Check sheet for the modelled part. Datum: model origin and axes. Units: mm. A direction names the side the tool comes from. Coordinates: 2 decimals unless noted, no trailing zeros. Loops run counter-clockwise (first coordinate to the right, second up) from the corner with the lowest first, then second, coordinate; pieces in that order, holes last. Notation, with made-up numbers: (2, 5.25) - (8, 5.25) arc R15 ccw to (8, 12.25) - close; hole circle Ø9 at (89.5, -34.5). An arc over 180 degrees is marked (long way). Write each question's results on one line, items separated by ' | '. Start each with the question number.
1. Gauge pin test, flat ends, axial feed: P1, Ø5, axis at y = -1.5, z = 24, coming from the +X side; P2, Ø2, axis at x = 0.5, z = -4.5, coming from the +Y side; P3, Ø3, axis at y = 4, z = 42.5, coming from the -X side; P4, Ø1.5, axis at y = 2.5, z = 8.5, coming from the -X side. Record the tip position at first contact, or that the pin passes through.
2. Tool access check on faces 1 (the face through (3, 0, 38)), 2 (the face through (2.175, -1.233, -4.768)), 3 (the face through (1.08, 4.88, -2.71)). Record the directions out of +Z, -Z, +X, -X, +Y, -Y that give a thin tool (end or side, any length) a straight path to the whole face; none if there is none.
3. Thickness scan on line 1 (Z direction, x = 1.75, y = -3.25); line 2 (Z direction, x = -1.75, y = 0.25); line 3 (X direction, y = -0.25, z = 3). Record the ranges inside material, lowest first. Write a range as [from, to].
4. Cross-section at B-B (z = 12.5). Record the cut outline in (x, y).
```python
from build123d import *

# Parameters (mm, degrees)
CUT_EXTRUDE1_DEPTH = 2.5


with BuildPart() as part:
    # Logo3_bib1 → Revolve1 (revolve)
    with BuildSketch(Plane(origin=(0, 0, 0), x_dir=(-1, 0, 0), z_dir=(0, -1, 0))):
        with BuildLine():
            Line((0, -50), (0, 6))
            Line((0, 6), (4.5, 6))
            ThreePointArc((4.5, 6), (4.853553391, 5.853553391), (5, 5.5))
            Line((5, 5.5), (5, 0))
            Line((5, 0), (3, 0))
            Line((3, 0), (3, -26.01))
            Line((3, -26.01), (2.613425636, -26.01))
            ThreePointArc((2.613425636, -26.01), (2.593729481, -26.026527036), (2.606585234, -26.048793852))
            Line((2.606585234, -26.048793852), (3, -26.191985117))
            Line((3, -26.191985117), (3, -49.5))
            Line((3, -49.5), (2.5, -50))
            Line((2.5, -50), (0, -50))
        make_face()
    revolve(axis=Axis((0, 0, -10.585154653), (0, 0, 1)))

    # Logo3_bib2 → Cut-Extrude1 (cut)
    with BuildSketch(Plane(origin=(0, 0, -6), x_dir=(1, 0, 0), z_dir=(0, 0, -1))):
        Polygon((2.886751346, 0), (1.443375673, 2.5), (-1.443375673, 2.5), (-2.886751346, 0), (-1.443375673, -2.5), (1.443375673, -2.5), align=None)
    extrude(amount=-CUT_EXTRUDE1_DEPTH, mode=Mode.SUBTRACT)


solid = part.part
```
Established:
1) P1: x = 3 | P2: y = 5 | P3: x = -1.66 | P4: x = -2.44
2) face 1: +Z | face 2: -Z | face 3: +Z, -Z
3) line 1: [-6, 0] | line 2: [-3.5, 50] | line 3: [-2.99, 2.99]
4) outline: circle Ø6 at (0, 0)
